from build123d import *

# Parameters (mm, degrees)
SKETCH_1_R                  = 10
EXTRUDE_1_DEPTH             = 50
PATTERN_LINEAR_1_COUNT      = 2
PATTERN_LINEAR_1_PITCH      = 40
PATTERN_LINEAR_1_COUNT_DIR2 = 2
PATTERN_LINEAR_1_PITCH_DIR2 = 40


with BuildPart() as part:
    # 草图1 → 拉伸1 (new body)
    with BuildSketch(Plane.XY):
        Polygon((5, -20), (-5, -20), (-11, -14), (-25, -14), (-25, 8), (-27, 10), (-27, 21), (-13, 21), (-13, 19), (13, 19), (13, 21), (27, 21), (27, 10), (25, 8), (25, -14), (11, -14), align=None)
        Circle(SKETCH_1_R, mode=Mode.SUBTRACT)
    extrude(amount=EXTRUDE_1_DEPTH)

    # 草图2 → M6x1.0 螺纹孔1 (revolve, cut)
    with BuildSketch(Plane(origin=(20, 21, 5), x_dir=(0, 0, 1), z_dir=(1, 0, 0))):
        Polygon((0, 0), (0, 18.502151548), (2.5, 17), (2.5, 0), align=None)
    m6x1_0_1 = revolve(axis=Axis((20, 27.35, 5), (0, -1, 0)), mode=Mode.SUBTRACT)

    # 阵列(线性)1: M6x1.0 _1 2 × 2
    with Locations(*[(-j * PATTERN_LINEAR_1_PITCH_DIR2, 0, i * PATTERN_LINEAR_1_PITCH) for i in range(PATTERN_LINEAR_1_COUNT) for j in range(PATTERN_LINEAR_1_COUNT_DIR2) if (i, j) != (0, 0)]):
        add(m6x1_0_1, mode=Mode.SUBTRACT)


solid = part.part
Model file for the job. Use its own axes, mm. A direction names the side the tool comes from. Give positions to 0.01 mm unless a question says otherwise; leave off trailing zeros. Loops run counter-clockwise (first coordinate to the right, second up) from the corner with the lowest first, then second, coordinate; pieces in that order, holes last.
Item 1: Slice it at D-D (y = 0). Write the cut outline in (x, z).
Check values:
outline: (-25, 0) - (-10, 0) - (-10, 50) - (-25, 50) - close; (10, 0) - (25, 0) - (25, 50) - (10, 50) - close
Item 2: Which spindle directions (+Z, -Z, +X, -X, +Y, -Y) get a long thin tool onto all of the face, cutting with end or side? Do faces 4 (the face through (18, -14, 25)), 5 (the face through (-13, 20, 25)), 6 (the face through (-2.17, -9.76, 24.65)), 7 (the face through (-18, -14, 25)), 8 (the face through (-22.11, 12.62, 46.34)). Say none if no direction does.
Check values:
face 4: +Z, -Z, +X, -Y
face 5: +Z, -Z, +Y
face 6: +Z, -Z
face 7: +Z, -Z, -X, -Y
face 8: +Y
Item 3: Mould opens along Z. For faces 1 (the face through (-6, 10, 0)), 2 (the face through (0, -20, 25)), 3 (the face through (-20.019, 2.759, 4.566)) say: +Z half, -Z half, draft (parallel to the pull), parting line (faces both ways), or undercut.
Check values:
face 1: -Z half
face 2: draft
face 3: undercut
Item 4: Drop flat-ended pins along their axis: P1, Ø7, axis at x = 17, z = 18, coming from the -Y side; P2, Ø18, axis at x = 0, y = 0, coming from the +Z side; P3, Ø11, axis at y = 1, z = 35, coming from the -X side; P4, Ø1, axis at x = -7.5, z = 25, coming from the -Y side. Give the stop position or say it passes through.
Check values:
P1: stops at y = -14
P2: passes through
P3: stops at x = -25
P4: stops at y = -18
Item 5: Slice it at A-A (x = 0). Write the cut outline in (y, z).
Check values:
outline: (-20, 0) - (-10, 0) - (-10, 50) - (-20, 50) - close; (10, 0) - (19, 0) - (19, 50) - (10, 50) - close
Item 6: Slice it at B-B (z = 21). Write the cut outline in (x, y), plus the area to 3 significant figures.
Check values:
outline: (-27, 10) - (-25, 8) - (-25, -14) - (-11, -14) - (-5, -20) - (5, -20) - (11, -14) - (25, -14) - (25, 8) - (27, 10) - (27, 21) - (13, 21) - (13, 19) - (-13, 19) - (-13, 21) - (-27, 21) - close; hole circle Ø20 at (0, 0)
area: 1,530 mm2
Item 7: Drill centre lines: line 1 along X through (y, z) = (11, 45); line 2 along Z through (x, y) = (20, 16); line 3 along X through (y, z) = (-0.5, 22.5). Where is each one in solid material? Low to high.
Check values:
line 1: x = -27 to -22.5, -17.5 to 17.5, 22.5 to 27
line 2: z = 0 to 2.5, 7.5 to 42.5, 47.5 to 50
line 3: x = -25 to -9.99, 9.99 to 25
Item 8: Slice it at C-C (y = 11.5). Write the cut outline in (x, z), plus the area to 3 significant figures.
Check values:
outline: (-27, 0) - (27, 0) - (27, 50) - (-27, 50) - close; hole circle Ø5 at (-20, 5); hole circle Ø5 at (-20, 45); hole circle Ø5 at (20, 5); hole circle Ø5 at (20, 45)
area: 2,620 mm2
